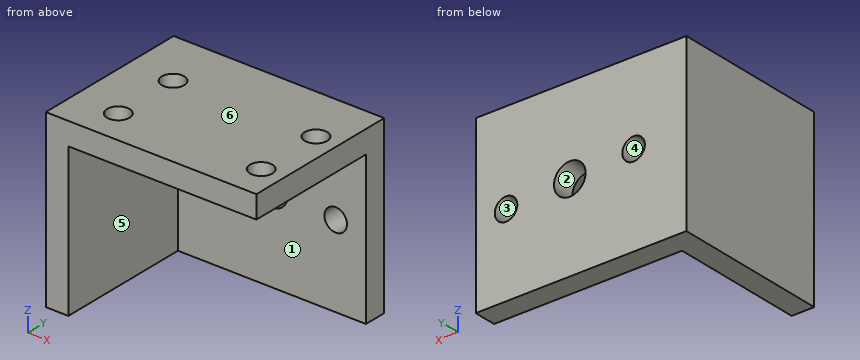
```python
from build123d import *

# Parameters (mm, degrees)
SKETCH1_W           = 25
SKETCH1_H           = 18
SKETCH1_R           = 1.5
BOSS_EXTRUDE1_DEPTH = 3
SKETCH2_W           = 25
SKETCH2_H           = 23
SKETCH2_R           = 2.1
SKETCH2_R_2         = 1.5
BOSS_EXTRUDE2_DEPTH = 3
SKETCH3_W           = 23
SKETCH3_H           = 21
BOSS_EXTRUDE3_DEPTH = 3


with BuildPart() as part:
    # Sketch1 → Boss-Extrude1 (new body)
    with BuildSketch(Plane.XY):
        Rectangle(SKETCH1_W, SKETCH1_H)
        with Locations((-9.5, 4.5)):
            Circle(SKETCH1_R, mode=Mode.SUBTRACT)
        with Locations((9.5, 4.5)):
            Circle(SKETCH1_R, mode=Mode.SUBTRACT)
        with Locations((9.5, -4.5)):
            Circle(SKETCH1_R, mode=Mode.SUBTRACT)
        with Locations((-9.5, -4.5)):
            Circle(SKETCH1_R, mode=Mode.SUBTRACT)
    extrude(amount=BOSS_EXTRUDE1_DEPTH)

    # Sketch2 → Boss-Extrude2 (add)
    with BuildSketch(Plane(origin=(0, 9, 0), x_dir=(1, 0, 0), z_dir=(0, 1, 0))):
        with Locations((0, 8.5)):
            Rectangle(SKETCH2_W, SKETCH2_H)
        with Locations(Location((0, 8.5, 0), (0, 0, 270))):
            Circle(SKETCH2_R, mode=Mode.SUBTRACT)
        with Locations(Location((-8.477677472, 7.884382628, 0), (0, 0, 270))):
            Circle(SKETCH2_R_2, mode=Mode.SUBTRACT)
        with Locations(Location((8.477677464, 9.115617375, 0), (0, 0, 270))):
            Circle(SKETCH2_R_2, mode=Mode.SUBTRACT)
    extrude(amount=BOSS_EXTRUDE2_DEPTH)

    # Sketch3 → Boss-Extrude3 (add)
    with BuildSketch(Plane.ZY.offset(12.5)):
        with Locations((-8.5, 1.5)):
            Rectangle(SKETCH3_W, SKETCH3_H)
    extrude(amount=BOSS_EXTRUDE3_DEPTH)


solid = part.part
```
For this review, take the finished solid that the model builds, in its own axes (mm). Face numbers are marked on the shaded views. A direction names the side the tool comes from. Round coordinates to 2 decimals unless told otherwise and drop trailing zeros. Loops run counter-clockwise (first coordinate to the right, second up) from the corner with the lowest first, then second, coordinate; pieces in that order, holes last.
(1) We need section D-D (x = 9.5). Give the boundary of the cut face in (y, z).
Returned:
outline: (-9, 0) - (-6, 0) - (-6, 3) - (-9, 3) - close; (-3, 0) - (3, 0) - (3, 3) - (-3, 3) - close; (6, 0) - (9, 0) - (9, -8.02) - (12, -8.02) - (12, 3) - (6, 3) - close; (9, -20) - (12, -20) - (12, -10.21) - (9, -10.21) - close
(2) Clearance check with flat-ended pins moving along their axes: P1, Ø5, axis at y = 5.5, z = -16, coming from the +X side; P2, Ø5, axis at x = -6, z = -3, coming from the -Y side; P3, Ø3.5, axis at x = 9.5, y = -4.5, coming from the +Z side; P4, Ø5.5, axis at x = -2, y = -2, coming from the -Z side. State where each tip first meets the part, or that it passes through.
Returned:
P1: stops at x = -12.5
P2: stops at y = 9
P3: stops at z = 3
P4: stops at z = 0
(3) We need section B-B (z = -8.5). Give the boundary of the cut face in (x, y).
Returned:
outline: (-15.5, -9) - (-12.5, -9) - (-12.5, 9) - (-9.85, 9) - (-9.85, 12) - (-15.5, 12) - close; (-7.11, 9) - (-2.1, 9) - (-2.1, 12) - (-7.11, 12) - close; (2.1, 9) - (7.11, 9) - (7.11, 12) - (2.1, 12) - close; (9.85, 9) - (12.5, 9) - (12.5, 12) - (9.85, 12) - close
(4) Mouldability with a two-part tool opening along Z and no side actions: class the marked faces 3, 4, 5 and 6 as released by +Z, released by -Z, zero draft, split by the parting line, or undercut.
Returned:
face 3: undercut
face 4: undercut
face 5: zero draft
face 6: released by +Z
(5) Tool access review of the marked faces 1 and 2: name each direction out of +Z, -Z, +X, -X, +Y, -Y from which nothing blocks a thin tool from reaching the whole face with its end or side.
Returned:
face 1: -Z, +X, -Y
face 2: +Y, -Y
(6) We need section C-C (y = -6.5). Give the boundary of the cut face in (x, z).
Returned:
outline: (-15.5, -20) - (-12.5, -20) - (-12.5, 0) - (12.5, 0) - (12.5, 3) - (-15.5, 3) - close
(7) Wall thickness on line 1 along Y through (x, z) = (-9.5, 1.7); line 2 along X through (y, z) = (9.9, -8.5); line 3 along X through (y, z) = (-3.25, -8): over which ranges is each line inside the solid? List them lowest first.
Returned:
line 1: y = -9 to -6, -3 to 3, 6 to 12
line 2: x = -15.5 to -9.85, -7.11 to -2.1, 2.1 to 7.11, 9.85 to 12.5
line 3: x = -15.5 to -12.5
(8) We need section A-A (x = 0). Give the boundary of the cut face in (y, z), plus the area to 3 significant figures.
Returned:
outline: (-9, 0) - (9, 0) - (9, -6.4) - (12, -6.4) - (12, 3) - (-9, 3) - close; (9, -20) - (12, -20) - (12, -10.6) - (9, -10.6) - close
area: 110 mm2
